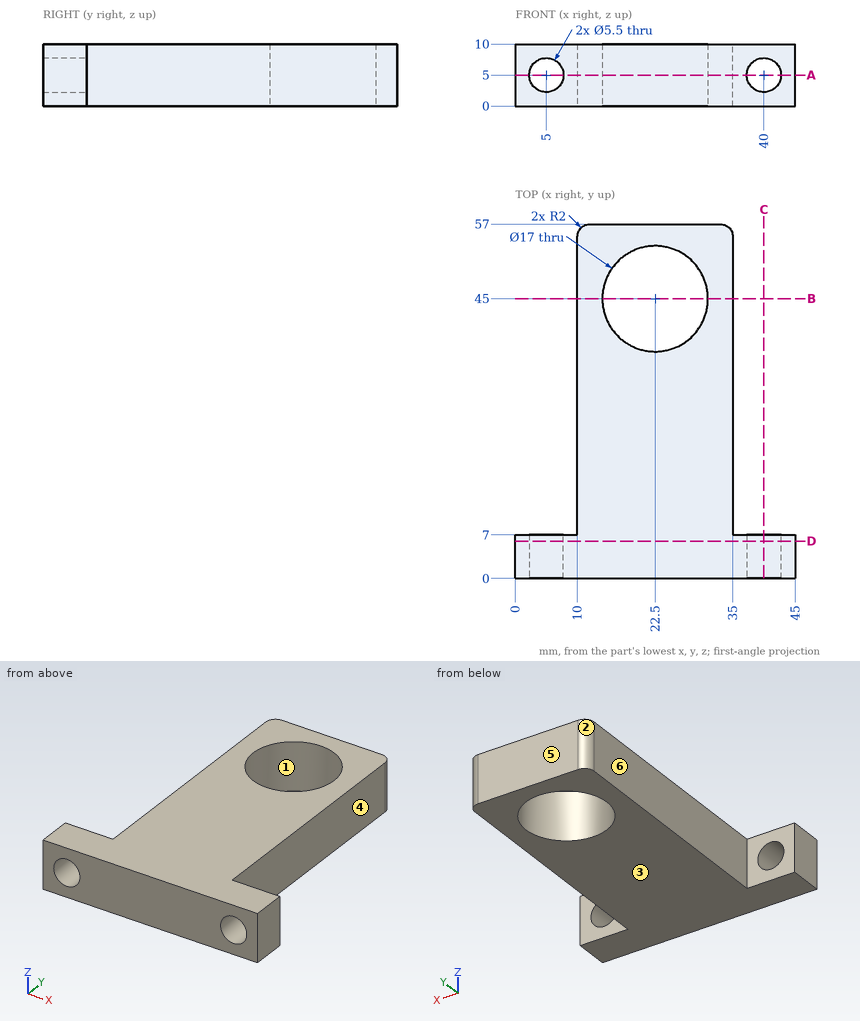
Check sheet for the drawn part. Datum: minimum x, y, z corner. Units: mm. A direction names the side the tool comes from. Round coordinates to 2 decimals unless told otherwise and drop trailing zeros. Order: outer loops, then holes, each group sorted by start corner. A loop starts at its lowest first (then second) coordinate and runs counter-clockwise, first axis right, second up. Notation, with made-up numbers: (-2, 83) -> (43, 83) arc R27 ccw to (43, 105) -> close; hole circle Ø6 at (55, 66). An arc over 180 degrees is marked (long way). Use CSV: the item, a comma, the result in double quotes.
(1) Cross-section at C-C (x = 40). Record the boundary of the cut face in (y, z).
Worked out:
outline,"(0, 0) -> (7, 0) -> (7, 2.25) -> (0, 2.25) -> close; (0, 7.75) -> (7, 7.75) -> (7, 10) -> (0, 10) -> close"
(2) Tool access check on the marked faces 4, 5 and 6. Record the directions out of +Z, -Z, +X, -X, +Y, -Y that give a thin tool (end or side, any length) a straight path to the whole face; none if there is none.
Worked out:
face 4,"+Z, -Z, +X, +Y"
face 5,"+Z, -Z, +X, -X, +Y"
face 6,"+Z, -Z, -X, +Y"
(3) Draft check along Y on the marked faces 1, 2 and 3. Enter one of: pulls with the +Y half, pulls with the -Y half, needs draft (parallel to the pull), parting line crosses it, or undercut.
Worked out:
face 1,"undercut"
face 2,"pulls with the +Y half"
face 3,"needs draft"
(4) Depth check by flat-ended pin: pin 1 (3 mm diameter, centred on y = 23.5, z = 2.5, fed in from +X); pin 2 (3 mm diameter, centred on x = 5.5, z = 7.5, fed in from +Y); pin 3 (10 mm diameter, centred on x = 22.5, y = 45, fed in from -Z); pin 4 (5 mm diameter, centred on y = 27, z = 8, fed in from -X). Enter the tip coordinate at first touch or a pass-through.
Worked out:
pin 1,"x = 35"
pin 2,"y = 7"
pin 3,"through"
pin 4,"x = 10"
(5) Cross-section at B-B (y = 45). Record the boundary of the cut face in (x, z).
Worked out:
outline,"(10, 0) -> (14, 0) -> (14, 10) -> (10, 10) -> close; (31, 0) -> (35, 0) -> (35, 10) -> (31, 10) -> close"
(6) Cross-section at A-A (z = 5). Record the boundary of the cut face in (x, y).
Worked out:
outline,"(0, 0) -> (2.25, 0) -> (2.25, 7) -> (0, 7) -> close; (7.75, 0) -> (37.25, 0) -> (37.25, 7) -> (35, 7) -> (35, 55) arc R2 ccw to (33, 57) -> (12, 57) arc R2 ccw to (10, 55) -> (10, 7) -> (7.75, 7) -> close; (42.75, 0) -> (45, 0) -> (45, 7) -> (42.75, 7) -> close; hole circle Ø17 at (22.5, 45)"
(7) Material ranges on line 1 along Z through (x, y) = (40, 4); line 2 along Y through (x, z) = (36, 6.25); line 3 along X through (y, z) = (51, 4), recorded low to high. Write a range as from..to.
Worked out:
line 1,"0..2.25, 7.75..10"
line 2,"0..7"
line 3,"10..16.48, 28.52..35"
(8) Cross-section at D-D (y = 6). Record the boundary of the cut face in (x, z), and give its area (3 significant figures).
Worked out:
outline,"(0, 0) -> (45, 0) -> (45, 10) -> (0, 10) -> close; hole circle Ø5.5 at (5, 5); hole circle Ø5.5 at (40, 5)"
area,"402 mm²"
